from build123d import *

# Parameters (mm, degrees)
SKETCH_1_W          = 600
SKETCH_1_H          = 150
EXTRUDE_1_DEPTH     = 14
SKETCH_2_W          = 600
SKETCH_2_H          = 25
CUT_EXTRUDE_1_DEPTH = 1.5
SKETCH_3_W          = 42
SKETCH_3_H          = 60
CUT_EXTRUDE_2_DEPTH = 1.5
FILLET_1_R          = 5


with BuildPart() as part:
    # 草图1 → 凸台-拉伸1 (new body)
    with BuildSketch(Plane.XY):
        Rectangle(SKETCH_1_W, SKETCH_1_H)
    extrude(amount=EXTRUDE_1_DEPTH)

    # 草图2 → 切除-拉伸1 (cut)
    with BuildSketch(Plane.XY.offset(14)):
        with Locations((0, 62.5)):
            Rectangle(SKETCH_2_W, SKETCH_2_H)
        with Locations((0, -62.5)):
            Rectangle(SKETCH_2_W, SKETCH_2_H)
    extrude(amount=-CUT_EXTRUDE_1_DEPTH, mode=Mode.SUBTRACT)

    # 草图3 → 切除-拉伸2 (cut)
    with BuildSketch(Plane.XY.offset(14)):
        with Locations((-279, 0)):
            Rectangle(SKETCH_3_W, SKETCH_3_H)
        with Locations((279, 0)):
            Rectangle(SKETCH_3_W, SKETCH_3_H)
    extrude(amount=-CUT_EXTRUDE_2_DEPTH, mode=Mode.SUBTRACT)

    # 圆角1
    fillet_1_edges = [part.edges().sort_by_distance(p)[0] for p in [
        (-258, 30, 13.25),
        (-258, -30, 13.25),
        (258, -30, 13.25),
        (258, 30, 13.25),
    ]]
    fillet(fillet_1_edges, radius=FILLET_1_R)


solid = part.part
Source: CAD feature listing. Evaluate the final solid. Frame: model axes, mm. A direction names the side the tool comes from. Round coordinates to 2 decimals unless told otherwise and drop trailing zeros. Loops run counter-clockwise (first coordinate to the right, second up) from the corner with the lowest first, then second, coordinate; pieces in that order, holes last.
Q1. Section B-B, the plane x = -231.5. Return loops of the section in (y, z), plus the area to 4 significant figures.
Q2. Mould query, pull axis Y, two halves, no side actions, for faces 6 (the face through (-4, -75, 6)), 7 (the face through (279, 0, 12.5)), 8 (the face through (-4, 1, 14)). Classes: pulls with the +Y half, pulls with the -Y half, needs draft (parallel to the pull), parting line crosses it, or undercut.
Q3. Section A-A, the plane y = 10.5. Return loops of the section in (x, z), plus the area to 3 significant figures.
Q4. Access query for faces 1 (the face through (300, -1, 7)), 2 (the face through (-300, -1, 7)), 3 (the face through (-4, -62, 12.5)), 4 (the face through (-279, 0, 12.5)), 5 (the face through (-4, 63, 12.5)). Directions: +Z, -Z, +X, -X, +Y, -Y. A direction counts if a zero-diameter tool reaches every point of the face in a straight line with its end or side. Return the directions, or none.
Q5. Section C-C, the plane y = -63. Return loops of the section in (x, z).
Q6. Ray query, line 1 (Z direction, x = 1.5, y = -56.5). Return the intervals inside material, ascending.
Q7. First-contact query: P1, Ø12.5, axis at x = -125, y = -64, coming from the +Z side; P2, Ø0.8, axis at x = -289, z = 13.5, coming from the -Y side; P3, Ø0.8, axis at x = 285.5, z = 13.5, coming from the +Y side. Flat tips, straight axial feed; report the tip coordinate or a pass-through.
Solutions:
1. outline: (-75, 0) - (75, 0) - (75, 12.5) - (50, 12.5) - (50, 14) - (-50, 14) - (-50, 12.5) - (-75, 12.5) - close
1. area: 2,025 mm2
2. face 6: pulls with the -Y half
2. face 7: undercut
2. face 8: needs draft
3. outline: (-300, 0) - (300, 0) - (300, 12.5) - (258, 12.5) - (258, 14) - (-258, 14) - (-258, 12.5) - (-300, 12.5) - close
3. area: 8,270 mm2
4. face 1: +Z, -Z, +X, +Y, -Y
4. face 2: +Z, -Z, -X, +Y, -Y
4. face 3: +Z, +X, -X, -Y
4. face 4: +Z, -X
4. face 5: +Z, +X, -X, +Y
5. outline: (-300, 0) - (300, 0) - (300, 12.5) - (-300, 12.5) - close
6. line 1: z = 0 to 12.5
7. P1: stops at z = 12.5
7. P2: stops at y = -50
7. P3: stops at y = 50
